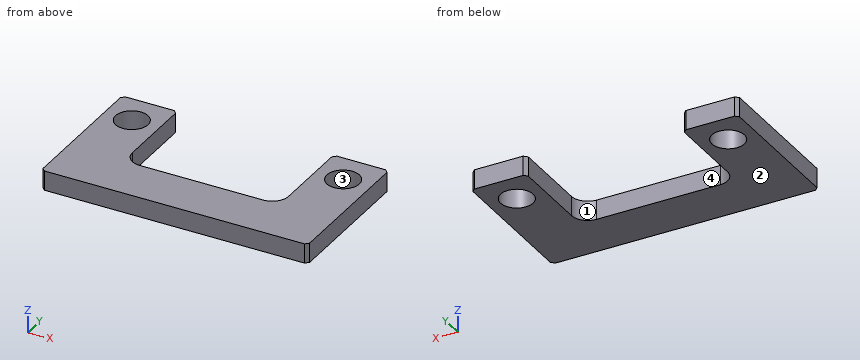
from build123d import *

# Parameters (mm, degrees)
SKETCH_1_R      = 10
EXTRUDE_1_DEPTH = 6
FILLET_1_R      = 10
CHAMFER_1_SIZE  = 2


with BuildPart() as part:
    # 草图1 → 凸台-拉伸1 (new, symmetric)
    with BuildSketch(Plane.XY):
        Polygon((-82, -70), (-82, 20), (-48, 20), (-48, -40), (48, -40), (48, 20), (82, 20), (82, -70), align=None)
        with Locations((-65, 0)):
            Circle(SKETCH_1_R, mode=Mode.SUBTRACT)
        with Locations((65, 0)):
            Circle(SKETCH_1_R, mode=Mode.SUBTRACT)
    extrude(amount=EXTRUDE_1_DEPTH, both=True)

    # 圆角1
    fillet_1_edges = [part.edges().sort_by_distance(p)[0] for p in [
        (-48, -40, 0),
        (48, -40, 0),
    ]]
    fillet(fillet_1_edges, radius=FILLET_1_R)

    # 倒角1
    chamfer_1_edges = [part.edges().sort_by_distance(p)[0] for p in [
        (-48, 20, 0),
        (48, 20, 0),
        (82, 20, 0),
        (82, -70, 0),
        (-82, -70, 0),
        (-82, 20, 0),
    ]]
    chamfer(chamfer_1_edges, length=CHAMFER_1_SIZE)


solid = part.part
Design review of the part built by this model. Coordinates are the model's own, in mm. Face numbers are marked on the shaded views. A direction names the side the tool comes from. Round coordinates to 2 decimals unless told otherwise and drop trailing zeros. Write each loop counter-clockwise with the first axis right and the second up, starting at its lowest first coordinate (ties: lowest second). Pieces come first, ordered by that corner, then holes. Notation, with made-up numbers: M 2.5,-29 L 60.5,-29 A11 ccw 60.5,-10 Z; hole C 85.5,33.5 d8. An arc over 180 degrees is marked long. One line per item, written item: value. Start each with the question number.
1. Take a section at D-D on y = 12. State the section outline as (x, z) points, then the cut area to 3 significant figures.
2. For the marked faces 3 and 4, list the 3-axis set-ups (+Z, -Z, +X, -X, +Y, -Y) from which the entire face can be reached by the end or side of a thin tool; tool diameter is ignored.
3. Take a section at B-B on y = 0. State the section outline as (x, z) points, then the cut area to 3 significant figures.
4. Draft analysis for pull direction X (two halves, no side actions). For the marked faces 1 and 2, state which applies: pulls with the +X half, pulls with the -X half, needs draft (parallel to the pull), parting line crosses it, or undercut.
5. Take a section at C-C on z = 0.25. State the section outline as (x, y) points, then the cut area to 3 significant figures.
6. To check wall thickness, follow probe 1 along Y at (x, z) = (-65, -1.25); probe 2 along X at (y, z) = (-7, 3); probe 3 along X at (y, z) = (-22.5, -4.75). State the ranges of each line that lie inside material, in increasing order. Write a range as from..to.
7. Clearance check with a flat-ended pin moving along its axis: P1, Ø1, axis at x = 19.5, z = 3.5, coming from the +Y side. State where the tip first meets the part, or that it passes through.
8. Take a section at A-A on x = 57. State the section outline as (y, z) points.
Computed:
1. outline: M -82,-6 L -48,-6 L -48,6 L -82,6 Z; M 48,-6 L 82,-6 L 82,6 L 48,6 Z
1. area: 816 mm²
2. face 3: +Z, -Z
2. face 4: +Z, -Z, +Y
3. outline: M -82,-6 L -75,-6 L -75,6 L -82,6 Z; M -55,-6 L -48,-6 L -48,6 L -55,6 Z; M 48,-6 L 55,-6 L 55,6 L 48,6 Z; M 75,-6 L 82,-6 L 82,6 L 75,6 Z
3. area: 336 mm²
4. face 1: undercut
4. face 2: needs draft
5. outline: M -82,-68 L -80,-70 L 80,-70 L 82,-68 L 82,18 L 80,20 L 50,20 L 48,18 L 48,-30 A10 cw 38,-40 L -38,-40 A10 cw -48,-30 L -48,18 L -50,20 L -80,20 L -82,18 Z; hole C -65,0 d20; hole C 65,0 d20
5. area: 8,400 mm²
6. probe 1: y = -70..-10, 10..20
6. probe 2: x = -82..-72.14, -57.86..-48, 48..57.86, 72.14..82
6. probe 3: x = -82..-48, 48..82
7. P1: stops at y = -40
8. outline: M -70,-6 L -6,-6 L -6,6 L -70,6 Z; M 6,-6 L 20,-6 L 20,6 L 6,6 Z
